Here's how the part is built. I have some questions about the finished solid (model axes, mm). A direction names the side the tool comes from. Coordinates: 2 decimals unless noted, no trailing zeros. Write each loop counter-clockwise with the first axis right and the second up, starting at its lowest first coordinate (ties: lowest second). Pieces come first, ordered by that corner, then holes.
Item 1: I want a section at C-C (z = -62). Please give me the cut outline in (x, y), and give its area (3 significant figures).
Item 2: I want a section at B-B (x = 17). Please give me the cut outline in (y, z).
Item 3: For faces 4 (the face through (0, 0, 0)), 5 (the face through (30.67, -0.53, -11.99)), 6 (the face through (94.016, 0.725, -97.269)), which set-ups out of +Z, -Z, +X, -X, +Y, -Y let a thin tool reach every point of the face, with its end or its side?
Item 4: Please list where these lines run through material, in increasing order: line 1 (X direction, y = -13.5, z = -202); line 2 (Z direction, x = 14, y = 4.5); line 3 (Z direction, x = 14.5, y = -4).
Item 5: I want a section at A-A (y = 0). Please give me the cut outline in (x, z).
Item 6: If we mould it in two halves opening along X, with no side actions, what happens to faces 1 (the face through (29, 12, -196)), 2 (the face through (98.51, -0.53, -131.24)), 3 (the face through (10, 0, -198))? For each: pulls with the +X half, pulls with the -X half, needs draft (parallel to the pull), parting line crosses it, or undercut.
Item 7: I'm going to push flat-ended pins straight in: P1, Ø2, axis at x = 99, z = -86.5, coming from the -Y side; P2, Ø4, axis at x = 91, y = -8.5, coming from the -Z side; P3, Ø10, axis at x = 111.5, y = -6, coming from the +Z side. Where does each tip first touch, or does it pass through?
from build123d import *

# Parameters (mm, degrees)
SWEEP_1_PROFILE_R = 12
EXTRUDE_START     = -14
SKETCH_14_R       = 14.5
EXTRUDE_1_DEPTH   = 5
SKETCH_16_R       = 16.5
EXTRUDE_2_DEPTH   = 16.5


with BuildPart() as part:
    # 扫描1: sweep along a path in 草图1
    with BuildLine(Plane(origin=(0, 0, 0), x_dir=(1, 0, 0), z_dir=(0, 1, 0))) as sweep_1_path:
        Line((0, 0), (60.5, 0))
        ThreePointArc((60.5, 0), (95.855339059, 14.644660941), (110.5, 50))
        Line((110.5, 50), (110.5, 148))
        ThreePointArc((110.5, 148), (95.855339059, 183.355339059), (60.5, 198))
        Line((60.5, 198), (10, 198))
    # 扫描1 profile (on start of the path) → 扫描1 (sweep)
    with BuildSketch(Plane(origin=(0, 0, 0), x_dir=(0, 0, 1), z_dir=(1, 0, 0))):
        Circle(SWEEP_1_PROFILE_R)
    sweep(path=sweep_1_path.line)

    # 草图14 → 凸台-拉伸1 (add)
    with BuildSketch(Plane.ZY.offset(-10).offset(EXTRUDE_START)):
        with Locations((-198, 0)):
            Circle(SKETCH_14_R)
    extrude(amount=-EXTRUDE_1_DEPTH)

    # 草图16 → 凸台-拉伸2 (add, symmetric)
    with BuildSketch(Plane.XY.offset(-97.5)):
        with Locations((110.5, 0)):
            Circle(SKETCH_16_R)
    extrude(amount=EXTRUDE_2_DEPTH, both=True)


solid = part.part
Answer:
1. outline: circle Ø24 at (110.5, 0)
1. area: 452 mm2
2. outline: circle Ø24 at (0, -198); circle Ø24 at (0, 0)
3. face 4: +Z, -Z, -X, +Y, -Y
3. face 5: -X
3. face 6: none
4. line 1: x = 24 to 29
4. line 2: z = -209.12 to -186.88, -11.12 to 11.12
4. line 3: z = -209.31 to -186.69, -11.31 to 11.31
5. outline: (0, -12) - (60.5, -12) arc R38 cw to (98.5, -50) - (98.5, -81) - (94, -81) - (94, -114) - (98.5, -114) - (98.5, -148) arc R38 cw to (60.5, -186) - (29, -186) - (29, -183.5) - (24, -183.5) - (24, -186) - (10, -186) - (10, -210) - (24, -210) - (24, -212.5) - (29, -212.5) - (29, -210) - (60.5, -210) arc R62 ccw to (122.5, -148) - (122.5, -114) - (127, -114) - (127, -81) - (122.5, -81) - (122.5, -50) arc R62 ccw to (60.5, 12) - (0, 12) - close
6. face 1: undercut
6. face 2: parting line crosses it
6. face 3: pulls with the -X half
7. P1: stops at y = -12.73
7. P2: stops at z = -200.15
7. P3: stops at z = -9.94
